```python
from build123d import *


with BuildPart() as part:
    # 草图1 → 旋转1 (revolve)
    with BuildSketch(Plane.XY, mode=Mode.PRIVATE) as revolve_1_sk:
        Polygon((-108.824631792, 0), (-108.824631792, 13), (-70.824631792, 13), (-70.824631792, 16), (-60.824631792, 16), (-60.824631792, 22), (-17.824631792, 22), (-17.824631792, 16), (562.175368208, 16), (562.175368208, 0), align=None)
    revolve(revolve_1_sk.sketch.rotate(Axis((-119.580443242, 0, 0), (1, 0, 0)), 90), axis=Axis((-119.580443242, 0, 0), (1, 0, 0)))


solid = part.part
```
Verification items for the finished model (mm, model axes). A direction names the side the tool comes from. Coordinates: 2 decimals unless noted, no trailing zeros. Write each loop counter-clockwise with the first axis right and the second up, starting at its lowest first coordinate (ties: lowest second). Pieces come first, ordered by that corner, then holes. Notation, with made-up numbers: (-23, -28) - (20, -28) arc R32 ccw to (20, 11) - close; hole circle Ø5 at (32, -24.75). An arc over 180 degrees is marked (long way). Write item = value, one per line.
Q1. Access from +Z, -Z, +X, -X, +Y, -Y to the whole of each face (thin tool, end or side, straight path). Record for faces 1 (the face through (-70.825, -13.1, 1.3)), 2 (the face through (-17.825, 16.2, 1.5)), 3 (the face through (562.175, 0, 0)).
Answer:
face_1 = -X
face_2 = +X
face_3 = +Z, -Z, +X, +Y, -Y
Q2. Material ranges on L1, parallel to X at y = -18.5, z = -7; L2, parallel to X at y = -14, z = -3; L3, parallel to Y at x = 343.5, z = 1.5, recorded low to high. Write a range as from..to.
Answer:
L1 = -60.82..-17.82
L2 = -70.82..562.18
L3 = -15.93..15.93
Q3. Cross-section at A-A (y = 0). Enter the section's corners in (x, z), plus the area to 3 significant figures.
Answer:
outline = (-108.82, -13) - (-70.82, -13) - (-70.82, -16) - (-60.82, -16) - (-60.82, -22) - (-17.82, -22) - (-17.82, -16) - (562.18, -16) - (562.18, 16) - (-17.82, 16) - (-17.82, 22) - (-60.82, 22) - (-60.82, 16) - (-70.82, 16) - (-70.82, 13) - (-108.82, 13) - close
area = 21,800 mm²
Q4. Cross-section at C-C (x = -52). Enter the section's corners in (y, z).
Answer:
outline = circle Ø44 at (0, 0)
Q5. Cross-section at D-D (x = 241). Enter the section's corners in (y, z).
Answer:
outline = circle Ø32 at (0, 0)
Q6. Go/stop test with flat-tipped pins: pin 1 Ø4 at (x, z) = (251, 12) entering from -Y; pin 2 Ø1.5 at (x, z) = (169.5, -5.5) entering from -Y; pin 3 Ø1 at (x, z) = (71.5, 13.5) entering from -Y. Record where each tip stops, or that it passes through.
Answer:
pin_1 = -12.49
pin_2 = -15.28
pin_3 = -9.33
